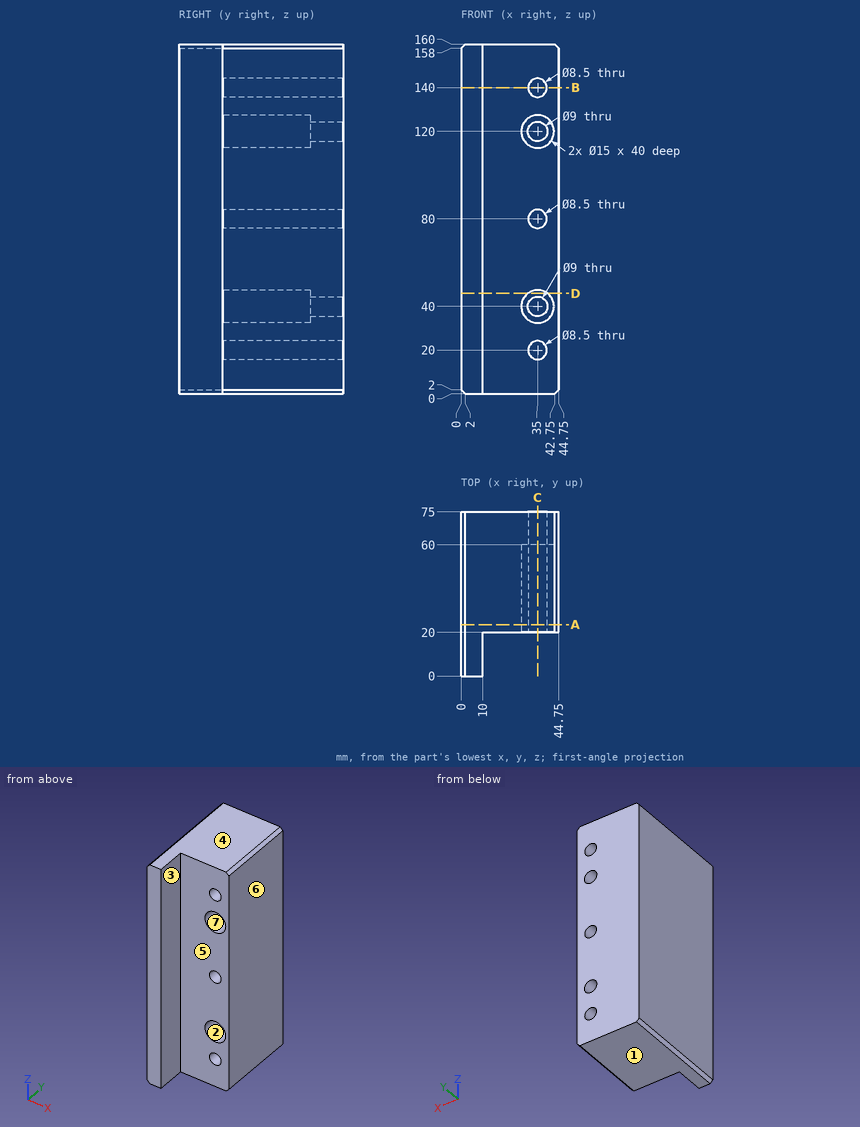
Geometry check sheet. Reference: drawing and pictorial views, mm from the part's lowest x, y, z. A direction names the side the tool comes from. Round coordinates to 2 decimals unless told otherwise and drop trailing zeros. Write each loop counter-clockwise with the first axis right and the second up, starting at its lowest first coordinate (ties: lowest second). Pieces come first, ordered by that corner, then holes. Notation, with made-up numbers: (-15.75, 63.5) -> (17.25, 63.5) arc R7 ccw to (17.25, 72.5) -> close; hole circle Ø9 at (-29, 78). An arc over 180 degrees is marked (long way). Answer as CSV lines item,"result". Start each with the question number.
1) Section check B-B on z = 140. Enter the section's corners in (x, y), and give its area (3 significant figures).
2) Tool access check on the marked faces 5, 6 and 7. Record the directions out of +Z, -Z, +X, -X, +Y, -Y that give a thin tool (end or side, any length) a straight path to the whole face; none if there is none.
3) Section check C-C on x = 35. State how many separate pieces and enclosed holes the cut face has, and give its area (3 significant figures).
4) Release check for a two-part mould opening along Z. For the marked faces 1, 2, 3 and 4 record: pulls with the +Z half, pulls with the -Z half, needs draft (parallel to the pull), parting line crosses it, or undercut.
5) Material ranges on line 1 (Z direction, x = 35, y = 65.75); line 2 (Z direction, x = 35, y = 51); line 3 (X direction, y = 13, z = 64.5), recorded low to high. Write a range as from..to.
6) Section check A-A on y = 23.5. Enter the section's corners in (x, z), and give its area (3 significant figures).
7) Section check D-D on z = 46. Enter the section's corners in (x, y).
8) Go/stop test with flat-tipped pins: P1, Ø12, axis at x = 39.5, z = 66.5, coming from the -Y side; P2, Ø4.5, axis at x = 34, z = 42.5, coming from the -Y side. Record where each tip stops, or that it passes through.
Found:
1,outline,"(0, 0) -> (10, 0) -> (10, 20) -> (30.75, 20) -> (30.75, 75) -> (0, 75) -> close; (39.25, 20) -> (44.75, 20) -> (44.75, 75) -> (39.25, 75) -> close"
1,area,"2,190 mm^2"
2,face 5,"+Z, -Z, +X, -Y"
2,face 6,"+Z, -Z, +X, +Y, -Y"
2,face 7,"-Y"
3,separate pieces,"6"
3,enclosed holes,"0"
3,area,"5,930 mm^2"
4,face 1,"pulls with the -Z half"
4,face 2,"undercut"
4,face 3,"needs draft"
4,face 4,"pulls with the +Z half"
5,line 1,"z = 0..15.75, 24.25..35.5, 44.5..75.75, 84.25..115.5, 124.5..135.75, 144.25..160"
5,line 2,"z = 0..15.75, 24.25..32.5, 47.5..75.75, 84.25..112.5, 127.5..135.75, 144.25..160"
5,line 3,"x = 0..10"
6,outline,"(0, 2) -> (2, 0) -> (42.75, 0) -> (44.75, 2) -> (44.75, 158) -> (42.75, 160) -> (2, 160) -> (0, 158) -> close; hole circle Ø15 at (35, 40); hole circle Ø15 at (35, 120); hole circle Ø8.5 at (35, 20); hole circle Ø8.5 at (35, 80); hole circle Ø8.5 at (35, 140)"
6,area,"6,630 mm^2"
7,outline,"(0, 0) -> (10, 0) -> (10, 20) -> (30.5, 20) -> (30.5, 60) -> (39.5, 60) -> (39.5, 20) -> (44.75, 20) -> (44.75, 75) -> (0, 75) -> close"
8,P1,"stops at y = 20"
8,P2,"stops at y = 60"
